from build123d import *

# Parameters (mm, degrees)
BASE_PLATE_SKETCH_W         = 142
BASE_PLATE_SKETCH_H         = 92
BASE_PLATE_142X92X14_DEPTH  = 14
BASE_CORNER_FILLETS_R10_R   = 10
BEARING_PEDESTAL_DEPTH      = 7.5
BEARING_BOSS_SKETCH_R       = 27.5
BEARING_BOSS_55_DEPTH       = 22.5
BORE_SKETCH_R               = 15
BORE_30_DEPTH               = 145.078103819
SUPPORT_RIB_1_REACH         = 132.603
SUPPORT_RIB_1_SKETCH_WALL_W = 303.284863468
SUPPORT_RIB_1_SKETCH_WALL_H = 15
SUPPORT_RIB_2_REACH         = 132.603
SUPPORT_RIB_2_SKETCH_WALL_W = 303.284863468
SUPPORT_RIB_2_SKETCH_WALL_H = 15
MOUNTING_HOLES_SKETCH_R     = 9
MOUNTING_HOLES_4X_18_DEPTH  = 41


with BuildPart() as part:
    # Base Plate Sketch → Base Plate 142x92x14 (new body)
    with BuildSketch(Plane(origin=(0, 0, 0), x_dir=(1, 0, 0), z_dir=(0, 1, 0))):
        Rectangle(BASE_PLATE_SKETCH_W, BASE_PLATE_SKETCH_H)
    extrude(amount=BASE_PLATE_142X92X14_DEPTH)

    # Base Corner Fillets R10
    base_corner_fillets_r10_edges = [part.edges().sort_by_distance(p)[0] for p in [
        (71, 7, 46),
        (-71, 7, 46),
        (-71, 7, -46),
        (71, 7, -46),
    ]]
    fillet(base_corner_fillets_r10_edges, radius=BASE_CORNER_FILLETS_R10_R)

    # Pedestal Sketch → Bearing Pedestal (add, symmetric)
    with BuildSketch(Plane(origin=(0, 0, 0), x_dir=(0, 0, -1), z_dir=(1, 0, 0))):
        Polygon((46, 14), (46, 36), (27.50046584, 72), (-27.49953416, 72), (-46, 36), (-46, 14), align=None)
    extrude(amount=BEARING_PEDESTAL_DEPTH, both=True)

    # Bearing Boss Sketch → Bearing Boss Ø55 (add, symmetric)
    with BuildSketch(Plane(origin=(0, 0, 0), x_dir=(0, 0, -1), z_dir=(1, 0, 0))):
        with Locations((0.00046584, 72)):
            Circle(BEARING_BOSS_SKETCH_R)
    extrude(amount=BEARING_BOSS_55_DEPTH, both=True)

    # Bore Sketch → Bore Ø30 (cut, through all)
    with BuildSketch(Plane(origin=(22.5, 0, 0), x_dir=(0, 0, -1), z_dir=(1, 0, 0))):
        with Locations((0.00046584, 72)):
            Circle(BORE_SKETCH_R)
    extrude(amount=-BORE_30_DEPTH, mode=Mode.SUBTRACT)

    # Support Rib 1 Sketch wall → Support Rib 1 (add, up to next)
    with BuildSketch(Plane(origin=(35.5, 29.25, 0), x_dir=(0.648734176014, -0.761015091093, 0), z_dir=(0.761015091093, 0.648734176014, 0)), mode=Mode.PRIVATE) as support_rib_1_sk1:
        Rectangle(SUPPORT_RIB_1_SKETCH_WALL_W, SUPPORT_RIB_1_SKETCH_WALL_H)
    support_rib_1_tool1 = extrude(support_rib_1_sk1.sketch, amount=-SUPPORT_RIB_1_REACH, mode=Mode.PRIVATE) - part.part
    add(support_rib_1_tool1.solids().sort_by_distance((35.5, 29.25, 0))[0])

    # Support Rib 2 Sketch wall → Support Rib 2 (add, up to next)
    with BuildSketch(Plane(origin=(-35.5, 29.25, 0), x_dir=(-0.648734176014, -0.761015091093, 0), z_dir=(0.761015091093, -0.648734176014, 0)), mode=Mode.PRIVATE) as support_rib_2_sk1:
        Rectangle(SUPPORT_RIB_2_SKETCH_WALL_W, SUPPORT_RIB_2_SKETCH_WALL_H)
    support_rib_2_tool1 = extrude(support_rib_2_sk1.sketch, amount=SUPPORT_RIB_2_REACH, mode=Mode.PRIVATE) - part.part
    add(support_rib_2_tool1.solids().sort_by_distance((-35.5, 29.25, 0))[0])

    # Mounting Holes Sketch → Mounting Holes 4xØ18 (cut)
    with BuildSketch(Plane(origin=(0, 14, 0), x_dir=(1, 0, 0), z_dir=(0, 1, 0))):
        with Locations(Location((-50, 25, 0), (0, 0, 270))):
            Circle(MOUNTING_HOLES_SKETCH_R)
        with Locations(Location((50, 25, 0), (0, 0, 270))):
            Circle(MOUNTING_HOLES_SKETCH_R)
        with Locations(Location((50, -25, 0), (0, 0, 270))):
            Circle(MOUNTING_HOLES_SKETCH_R)
        with Locations(Location((-50, -25, 0), (0, 0, 270))):
            Circle(MOUNTING_HOLES_SKETCH_R)
    extrude(amount=-MOUNTING_HOLES_4X_18_DEPTH, mode=Mode.SUBTRACT)


solid = part.part
Source: CAD feature listing. Evaluate the final solid. Frame: model axes, mm. A direction names the side the tool comes from. Round coordinates to 2 decimals unless told otherwise and drop trailing zeros. Order: outer loops, then holes, each group sorted by start corner. A loop starts at its lowest first (then second) coordinate and runs counter-clockwise, first axis right, second up. Notation, with made-up numbers: (53.25, -16.75) - (105.25, -16.75) arc R25 cw to (105.25, 2.25) - close; hole circle Ø3 at (-10, -27). An arc over 180 degrees is marked (long way). Use a Markdown table: item, result. Add a question column.
1. First-contact query: pin 1 (12 mm diameter, centred on x = 56, y = 25.5, fed in from +Z); pin 2 (25 mm diameter, centred on x = -23, y = 30.5, fed in from +Z); pin 3 (2 mm diameter, centred on y = 79.5, z = 21, fed in from +X); pin 4 (19.5 mm diameter, centred on y = 38.5, z = -23, fed in from -X). Flat tips, straight axial feed; report the tip coordinate or a pass-through.
2. Section query B-B (x = -13.5). Return the cut outline in (y, z), then the cut area to 3 significant figures.
3. Mould query, pull axis Y, two halves, no side actions, for faces 4 (the flat face through (0.11, 53.75, -36.88)), 5 (the flat face through (-22.5, 60, -12)), 6 (the flat face through (7.5, 37, -26)). Classes: +Y half, -Y half, draft (parallel to the pull), parting line (faces both ways), or undercut.
4. Section query D-D (x = 53.5). Return the cut outline in (y, z), then the cut area to 3 significant figures.
5. Set-up query: faces 1 (the flat face through (-7.5, 37, -26)), 2 (the flat face through (-23, 26, 7.5)), 3 (the flat face through (23, 26, 7.5)). Return all of +Z, -Z, +X, -X, +Y, -Y with unobstructed straight access to the full face (end or side cutting, diameter ignored); none if empty.
6. Section query C-C (z = 30). Return the cut outline in (x, y), then the cut area to 3 significant figures.
7. Section query A-A (z = 9.5). Return the cut outline in (x, y).
8. Line query: probe 1 along X at (y, z) = (7, -25); probe 2 along X at (y, z) = (9.5, 22); probe 3 along Y at (x, z) = (9, -30.5). Output: solid intervals per line, ascending.
Derived:
| question | item | result |
|---|---|---|
| 1 | pin 1 | through |
| 1 | pin 2 | z = 7.5 |
| 1 | pin 3 | x = 22.5 |
| 1 | pin 4 | x = -7.5 |
| 2 | outline | (0, -46) - (14, -46) - (14, -7.5) - (45.54, -7.5) arc R27.5 ccw (long way) to (45.54, 7.5) - (14, 7.5) - (14, 46) - (0, 46) - close; hole circle Ø30 at (72, 0) |
| 2 | area | 3,420 mm2 |
| 3 | face 4 | +Y half |
| 3 | face 5 | draft |
| 3 | face 6 | undercut |
| 4 | outline | (0, -46) - (14, -46) - (14, -33.29) - (0, -33.29) - close; (0, -16.71) - (14, -16.71) - (14, 16.71) - (0, 16.71) - close; (0, 33.29) - (14, 33.29) - (14, 46) - (0, 46) - close |
| 4 | area | 824 mm2 |
| 5 | face 1 | -Z, -X |
| 5 | face 2 | +Z, -X |
| 5 | face 3 | +Z, +X |
| 6 | outline | (-71, 0) - (-57.48, 0) - (-57.48, 14) - (-71, 14) - close; (-42.52, 0) - (42.52, 0) - (42.52, 14) - (7.5, 14) - (7.5, 67.13) - (-7.5, 67.13) - (-7.5, 14) - (-42.52, 14) - close; (57.48, 0) - (71, 0) - (71, 14) - (57.48, 14) - close |
| 6 | area | 2,370 mm2 |
| 7 | outline | (-71, 0) - (71, 0) - (71, 14) - (7.5, 14) - (7.5, 46.19) - (22.5, 46.19) - (22.5, 60.39) - (-22.5, 60.39) - (-22.5, 46.19) - (-7.5, 46.19) - (-7.5, 14) - (-71, 14) - close; (-22.5, 83.61) - (22.5, 83.61) - (22.5, 97.81) - (-22.5, 97.81) - close |
| 8 | probe 1 | -71 to -59, -41 to 41, 59 to 71 |
| 8 | probe 2 | -71 to -58.49, -41.51 to 41.51, 58.49 to 71 |
| 8 | probe 3 | 0 to 14 |
